```python
from build123d import *

# Parameters (mm, degrees)
SKETCH_1_W      = 50
SKETCH_1_H      = 200
SKETCH_1_R      = 6.5
EXTRUDE_1_DEPTH = 10


with BuildPart() as part:
    # 草图1 → 凸台-拉伸1 (new body)
    with BuildSketch(Plane.XY):
        Rectangle(SKETCH_1_W, SKETCH_1_H)
        with Locations((0, 80)):
            Circle(SKETCH_1_R, mode=Mode.SUBTRACT)
        with Locations((0, -80)):
            Circle(SKETCH_1_R, mode=Mode.SUBTRACT)
    extrude(amount=EXTRUDE_1_DEPTH)


solid = part.part
```
Here's how the part is built. I have some questions about the finished solid (model axes, mm). Coordinates: 2 decimals unless noted, no trailing zeros. Loops run counter-clockwise (first coordinate to the right, second up) from the corner with the lowest first, then second, coordinate; pieces in that order, holes last. Notation, with made-up numbers: (-5, -36.75) - (41, -36.75) arc R19 ccw to (41, -30.75) - close; hole circle Ø2 at (52, 41). An arc over 180 degrees is marked (long way). Return JSON: item names as keys, results as strings. Group by question number.
Item 1: We'd pull the mould along Y, two halves only. Please class faces 1 (the face through (-1.409, -86.345, 4.93)), 2 (the face through (0, -100, 5)), 3 (the face through (0, 100, 5)): +Y half, -Y half, draft (parallel to the pull), parting line (faces both ways), or undercut.
Item 2: If we section it at C-C on z = 8: Write out the boundary of the cut face in (x, y).
Item 3: If we section it at B-B on y = 80: Write out the boundary of the cut face in (x, z).
Item 4: If we section it at A-A on x = 0: Write out the boundary of the cut face in (y, z).
Item 5: I need wall thicknesses on line 1 (Y direction, x = 0, z = 6.5); line 2 (Y direction, x = 3, z = 9.75); line 3 (X direction, y = 83.5, z = 9.5). Which ranges of each line are inside material? Lowest first, please. Write a range as from..to.
Item 6: Will these pins go through, and if not, where does the flat tip stop? P1, Ø11.5, axis at x = 0, y = -80, coming from the -Z side; P2, Ø17, axis at x = 0, y = 80, coming from the -Z side.
Calculated:
{
 "1": {"face 1": "undercut", "face 2": "-Y half", "face 3": "+Y half"},
 "2": {"outline": "(-25, -100) - (25, -100) - (25, 100) - (-25, 100) - close; hole circle Ø13 at (0, -80); hole circle Ø13 at (0, 80)"},
 "3": {"outline": "(-25, 0) - (-6.5, 0) - (-6.5, 10) - (-25, 10) - close; (6.5, 0) - (25, 0) - (25, 10) - (6.5, 10) - close"},
 "4": {"outline": "(-100, 0) - (-86.5, 0) - (-86.5, 10) - (-100, 10) - close; (-73.5, 0) - (73.5, 0) - (73.5, 10) - (-73.5, 10) - close; (86.5, 0) - (100, 0) - (100, 10) - (86.5, 10) - close"},
 "5": {"line 1": "y = -100..-86.5, -73.5..73.5, 86.5..100", "line 2": "y = -100..-85.77, -74.23..74.23, 85.77..100", "line 3": "x = -25..-5.48, 5.48..25"},
 "6": {"P1": "passes through", "P2": "stops at z = 0"}
}
